```python
from build123d import *

# Parameters (mm, degrees)
SKETCH_2_W          = 4
SKETCH_2_H          = 6.8
CUT_EXTRUDE_1_DEPTH = 32.272991542


with BuildPart() as part:
    # 草图1 → 旋转1 (revolve)
    with BuildSketch(Plane.XY, mode=Mode.PRIVATE) as revolve_1_sk:
        Polygon((0, 5), (20, 5), (20, 8), (19, 8), (19, 15), (20, 15), (20, 17), (14.5, 17), (14.5, 8.5), (2, 8.5), (2, 7.9), (0.9, 7.9), (0.9, 8.5), (0, 8.5), align=None)
    revolve(revolve_1_sk.sketch.rotate(Axis((0, 0, 0), (1, 0, 0)), 90), axis=Axis((0, 0, 0), (1, 0, 0)))

    # 草图2 → 切除-拉伸1 (cut, through all)
    with BuildSketch(Plane(origin=(20, 0, 0), x_dir=(0, 0, -1), z_dir=(1, 0, 0))):
        with Locations((0, 3.4)):
            Rectangle(SKETCH_2_W, SKETCH_2_H)
    extrude(amount=-CUT_EXTRUDE_1_DEPTH, mode=Mode.SUBTRACT)


solid = part.part
```
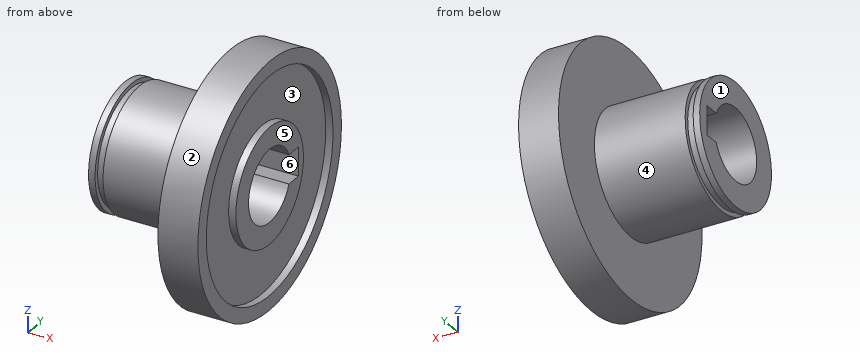
Geometry check sheet. Reference: the model listing, model coordinates, mm. Face numbers are marked on the shaded views. A direction names the side the tool comes from. Round coordinates to 2 decimals unless told otherwise and drop trailing zeros. Order: outer loops, then holes, each group sorted by start corner. A loop starts at its lowest first (then second) coordinate and runs counter-clockwise, first axis right, second up. Notation, with made-up numbers: M -32,64.5 L -20,64.5 A28 ccw -20,84.5 Z; hole C -38.5,55 d10. An arc over 180 degrees is marked long. Answer as CSV lines item,"result".
1) Mould release check, pull along Y, two halves, no side actions. Record for the marked faces 1, 2 and 3: +Y half, -Y half, draft (parallel to the pull), parting line (faces both ways), or undercut.
Entries:
face 1,"draft"
face 2,"parting line"
face 3,"undercut"
2) Sectioned sample at A-A on z = 0. Record the cut outline in (x, y), and give its area (3 significant figures).
Entries:
outline,"M 0,-8.5 L 0.9,-8.5 L 0.9,-7.9 L 2,-7.9 L 2,-8.5 L 14.5,-8.5 L 14.5,-17 L 20,-17 L 20,-15 L 19,-15 L 19,-8 L 20,-8 L 20,-5 L 0,-5 Z; M 0,6.8 L 20,6.8 L 20,8 L 19,8 L 19,15 L 20,15 L 20,17 L 14.5,17 L 14.5,8.5 L 2,8.5 L 2,7.9 L 0.9,7.9 L 0.9,8.5 L 0,8.5 Z"
area,"182 mm2"
3) Thickness scan on probe 1 along Y at (x, z) = (19.45, 0); probe 2 along Y at (x, z) = (10.5, 0); probe 3 along X at (y, z) = (-7, -15). Record the ranges inside material, lowest first. Write a range as [from, to].
Entries:
probe 1,"[-17, -15], [-8, -5], [6.8, 8], [15, 17]"
probe 2,"[-8.5, -5], [6.8, 8.5]"
probe 3,"[14.5, 20]"
4) Gauge pin test, flat ends, axial feed: pin 1 Ø4.5 at (x, z) = (12, 0) entering from -Y; pin 2 Ø1.5 at (x, z) = (18, -8.5) entering from +Y; pin 3 Ø10 at (x, z) = (3, 0.5) entering from +Y. Record the tip position at first contact, or that the pin passes through.
Entries:
pin 1,"y = -8.5"
pin 2,"y = 15.13"
pin 3,"y = 8.5"
5) Sectioned sample at B-B on y = 0. Record the cut outline in (x, z), and give its area (3 significant figures).
Entries:
outline,"M 0,-8.5 L 0.9,-8.5 L 0.9,-7.9 L 2,-7.9 L 2,-8.5 L 14.5,-8.5 L 14.5,-17 L 20,-17 L 20,-15 L 19,-15 L 19,-8 L 20,-8 L 20,-5 L 0,-5 Z; M 0,5 L 20,5 L 20,8 L 19,8 L 19,15 L 20,15 L 20,17 L 14.5,17 L 14.5,8.5 L 2,8.5 L 2,7.9 L 0.9,7.9 L 0.9,8.5 L 0,8.5 Z"
area,"218 mm2"
6) Tool access check on the marked faces 4, 5 and 6. Record the directions out of +Z, -Z, +X, -X, +Y, -Y that give a thin tool (end or side, any length) a straight path to the whole face; none if there is none.
Entries:
face 4,"-X"
face 5,"+Z, -Z, +X, +Y, -Y"
face 6,"+X, -X"
7) Sectioned sample at D-D on z = -12. Record the cut outline in (x, y), and give its area (3 significant figures).
Entries:
outline,"M 14.5,-12.04 L 20,-12.04 L 20,-9 L 19,-9 L 19,9 L 20,9 L 20,12.04 L 14.5,12.04 Z"
area,"114 mm2"
8) Sectioned sample at C-C on x = 18. Record the cut outline in (y, z), and give its area (3 significant figures).
Entries:
outline,"C 0,0 d34; hole M 4.58,-2 L 6.8,-2 L 6.8,2 L 4.58,2 A5 ccw long Z"
area,"822 mm2"
